Check sheet for the drawn part. Datum: minimum x, y, z corner. Units: mm. A direction names the side the tool comes from. Give positions to 0.01 mm unless a question says otherwise; leave off trailing zeros. Loops run counter-clockwise (first coordinate to the right, second up) from the corner with the lowest first, then second, coordinate; pieces in that order, holes last.
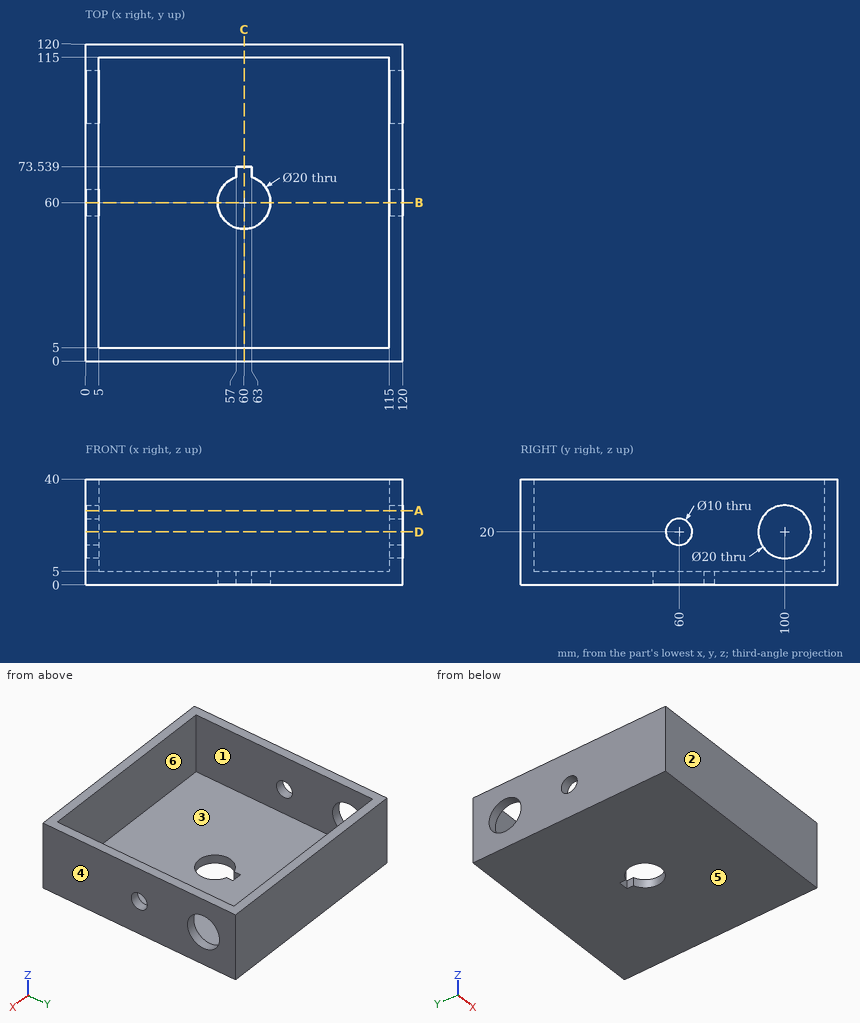
(1) Section check D-D on z = 20. Record the boundary of the cut face in (x, y).
(2) Section check B-B on y = 60. Record the boundary of the cut face in (x, z), plus the area to 3 significant figures.
(3) Release check for a two-part mould opening along X. For the marked faces 3, 4, 5 and 6 record: pulls with the +X half, pulls with the -X half, needs draft (parallel to the pull), parting line crosses it, or undercut.
(4) Section check C-C on x = 60. Record the boundary of the cut face in (y, z).
(5) Gauge pin test, flat ends, axial feed: pin 1 Ø4 at (x, y) = (97, 95.5) entering from -Z; pin 2 Ø1.5 at (x, y) = (36, 32.5) entering from +Z; pin 3 Ø12 at (y, z) = (100, 20) entering from +X. Record the tip position at first contact, or that the pin passes through.
(6) Section check A-A on z = 28. Record the boundary of the cut face in (x, y).
(7) Access from +Z, -Z, +X, -X, +Y, -Y to the whole of each face (thin tool, end or side, straight path). Record for the marked faces 1 and 2.
(8) Material ranges on line 1 (Y direction, x = 2, z = 20); line 2 (X direction, y = 110.5, z = 32), recorded low to high.
Computed values:
1. outline: (0, 0) - (120, 0) - (120, 55) - (115, 55) - (115, 5) - (5, 5) - (5, 55) - (0, 55) - close; (0, 65) - (5, 65) - (5, 90) - (0, 90) - close; (0, 110) - (5, 110) - (5, 115) - (115, 115) - (115, 110) - (120, 110) - (120, 120) - (0, 120) - close; (115, 65) - (120, 65) - (120, 90) - (115, 90) - close
2. outline: (0, 0) - (50, 0) - (50, 5) - (5, 5) - (5, 15) - (0, 15) - close; (0, 25) - (5, 25) - (5, 40) - (0, 40) - close; (70, 0) - (120, 0) - (120, 15) - (115, 15) - (115, 5) - (70, 5) - close; (115, 25) - (120, 25) - (120, 40) - (115, 40) - close
2. area: 750 mm2
3. face 3: undercut
3. face 4: pulls with the +X half
3. face 5: needs draft
3. face 6: undercut
4. outline: (0, 0) - (50, 0) - (50, 5) - (5, 5) - (5, 40) - (0, 40) - close; (73.54, 0) - (120, 0) - (120, 40) - (115, 40) - (115, 5) - (73.54, 5) - close
5. pin 1: stops at z = 0
5. pin 2: stops at z = 5
5. pin 3: passes through
6. outline: (0, 0) - (120, 0) - (120, 94) - (115, 94) - (115, 5) - (5, 5) - (5, 94) - (0, 94) - close; (0, 106) - (5, 106) - (5, 115) - (115, 115) - (115, 106) - (120, 106) - (120, 120) - (0, 120) - close
7. face 1: +Z
7. face 2: +Z, -Z, +X, -X, -Y
8. line 1: y = 0 to 55, 65 to 90, 110 to 120
8. line 2: x = 0 to 5, 115 to 120
